Could you check a few things on this model? Use its own coordinates, in mm. A direction names the side the tool comes from. Coordinates: 2 decimals unless noted, no trailing zeros. Write each loop counter-clockwise with the first axis right and the second up, starting at its lowest first coordinate (ties: lowest second). Pieces come first, ordered by that corner, then holes.
Item 1: Thinking about a two-plate mould opening in Y: for faces 1 (the flat face through (26, 0, 25)), 2 (the flat face through (54.84, 35.87, 25.07)), 3 (the flat face through (5.823, 38.787, 24.93)), 4 (the flat face through (26, 54, 10)), which applies, +Y half, -Y half, draft (parallel to the pull), parting line (faces both ways), or undercut?
Item 2: I want a section at D-D on z = 13. Please give me the cut outline in (x, y), then the cut area to 4 significant figures.
Item 3: For P1, Ø1, axis at x = 23, z = 23, coming from the +Y side; P2, Ø4, axis at x = -9.5, z = 11, coming from the -Y side; P3, Ø4.5, axis at x = -5.5, y = 42, coming from the +Z side, each with a flat end and sliding along its axis, tell me the tip position at first contact or that it passes through.
Item 4: I want a section at B-B on x = 26. Please give me the cut outline in (y, z), then the cut area to 3 significant figures.
Item 5: If I drill on probe 1 along Z at (x, y) = (6, 42.5); probe 2 along Y at (x, z) = (50.5, 10.5); probe 3 along Y at (x, z) = (56.5, 13), over which ranges is the centre line in solid material (lowest first)?
Item 6: I want a section at A-A on z = 25. Please give me the cut outline in (x, y), then the cut area to 3 significant figures.
Item 7: I want a section at C-C on y = 32.5. Please give me the cut outline in (x, z), then the cut area to 3 significant figures.
Item 8: Which directions (+Z, -Z, +X, -X, +Y, -Y) give clear straight access to the entire face, cutting with the end or side of a thin tool? Please do faces 5 (the flat face through (26, 45, 25)), 6 (the flat face through (56, 34, 7)), 7 (the cylindrical face through (26, 45, 45)), 8 (the flat face through (-2.84, 35.87, 24.93)), 9 (the flat face through (3.5, 47, 43)).
from build123d import *

# Parameters (mm, degrees)
BASE_BLOCK_DEPTH        = 50
SADDLE_CUT_1_30_DEPTH   = 10
SADDLE_START            = -10
SADDLE_CUT_2_30_DEPTH   = 10
UPPER_BLOCK_DEPTH       = 30
UPPER_BLOCK_NOTCH_DEPTH = 20
NOTCH_PAD_1_DEPTH       = 5
NOTCH_PAD_2_DEPTH       = 5
SIDE_BLOCK_DEPTH        = 35
SIDE_BLOCK_POCKET_DEPTH = 15
TOP_HOLE_SKETCH_R       = 5
TOP_HOLE_10_DEPTH       = 15
SIDE_WINDOW_SKETCH_W    = 10
SIDE_WINDOW_SKETCH_H    = 10
SIDE_WINDOW_CUT_DEPTH   = 15
UPPER_WINDOW_SKETCH_W   = 10
UPPER_WINDOW_SKETCH_H   = 10
UPPER_WINDOW_CUT_DEPTH  = 15


with BuildPart() as part:
    # Base Profile Sketch → Base Block (new body)
    with BuildSketch(Plane.XY):
        Polygon((0, 0), (52, 0), (52, 12), (71, 12), (71, 22), (63, 34), (48, 34), (48, 60), (4, 60), (4, 34), (-11, 34), (-19, 22), (-19, 12), (0, 12), align=None)
    extrude(amount=BASE_BLOCK_DEPTH)

    # Saddle Cut 1 Sketch → Saddle Cut 1 Ø30 (cut)
    with BuildSketch(Plane.XY.offset(50)):
        with BuildLine():
            Line((11, 60), (41, 60))
            ThreePointArc((41, 60), (26, 45), (11, 60))
        make_face()
    extrude(amount=-SADDLE_CUT_1_30_DEPTH, mode=Mode.SUBTRACT)

    # Saddle Cut 2 Sketch → Saddle Cut 2 Ø30 (cut)
    with BuildSketch(Plane(origin=(0, 0, 0), x_dir=(-1, 0, 0), z_dir=(0, 0, -1)).offset(SADDLE_START)):
        with BuildLine():
            Line((-41, 60), (-11, 60))
            ThreePointArc((-11, 60), (-26, 45), (-41, 60))
        make_face()
    extrude(amount=SADDLE_CUT_2_30_DEPTH, mode=Mode.SUBTRACT)

    # Upper Block Sketch → Upper Block (add)
    with BuildSketch(Plane(origin=(0, 0, 0), x_dir=(-1, 0, 0), z_dir=(0, 0, -1))):
        Polygon((-48, 60), (-48, 34), (-63, 34), (-56, 60), align=None)
    extrude(amount=-UPPER_BLOCK_DEPTH)

    # Upper Block Notch Sketch → Upper Block Notch (cut)
    with BuildSketch(Plane(origin=(0, 0, 0), x_dir=(-1, 0, 0), z_dir=(0, 0, -1))):
        Polygon((-63, 34), (-56, 60), (-48.5, 60), (-48.5, 34), align=None)
    extrude(amount=-UPPER_BLOCK_NOTCH_DEPTH, mode=Mode.SUBTRACT)

    # Notch Pad 1 Sketch → Notch Pad 1 (add)
    with BuildSketch(Plane(origin=(0, 0, 20), x_dir=(-1, 0, 0), z_dir=(0, 0, -1))):
        Polygon((-63, 34), (-48.5, 34), (-48.5, 60), (-56, 60), align=None)
    extrude(amount=NOTCH_PAD_1_DEPTH)

    # Notch Pad 2 Sketch → Notch Pad 2 (add)
    with BuildSketch(Plane.XY.offset(30)):
        Polygon((48, 60), (56, 60), (63, 34), (48, 34), align=None)
    extrude(amount=NOTCH_PAD_2_DEPTH)

    # Side Block Sketch → Side Block (add)
    with BuildSketch(Plane.XY.offset(50)):
        Polygon((4, 60), (4, 34), (-11, 34), (-4, 60), align=None)
    extrude(amount=-SIDE_BLOCK_DEPTH)

    # Side Block Pocket Sketch → Side Block Pocket (cut)
    with BuildSketch(Plane.XY.offset(50)):
        Polygon((3.5, 60), (3.5, 34), (-11, 34), (-4, 60), align=None)
    extrude(amount=-SIDE_BLOCK_POCKET_DEPTH, mode=Mode.SUBTRACT)

    # Top Hole Sketch → Top Hole Ø10 (cut)
    with BuildSketch(Plane(origin=(0, 60, 0), x_dir=(1, 0, 0), z_dir=(0, 1, 0))):
        with Locations(Location((26, -25, 0), (0, 0, 270))):
            Circle(TOP_HOLE_SKETCH_R)
    extrude(amount=-TOP_HOLE_10_DEPTH, mode=Mode.SUBTRACT)

    # Side Window Sketch → Side Window Cut (cut)
    with BuildSketch(Plane(origin=(-18.791724138, 5.059310345, 0), x_dir=(0, 0, 1), z_dir=(-0.9656157585206698, 0.25997347344787275, 0))):
        with Locations((25, 38.897051617)):
            Rectangle(SIDE_WINDOW_SKETCH_W, SIDE_WINDOW_SKETCH_H)
    extrude(amount=-SIDE_WINDOW_CUT_DEPTH, mode=Mode.SUBTRACT)

    # Upper Window Sketch → Upper Window Cut (cut)
    with BuildSketch(Plane(origin=(67.277241379, 18.113103448, 0), x_dir=(0, 0, -1), z_dir=(0.9656157585206697, 0.2599734734478728, 0))):
        with Locations((-25, 25.378430998)):
            Rectangle(UPPER_WINDOW_SKETCH_W, UPPER_WINDOW_SKETCH_H)
    extrude(amount=-UPPER_WINDOW_CUT_DEPTH, mode=Mode.SUBTRACT)


solid = part.part
Response values:
1. face 1: -Y half
1. face 2: undercut
1. face 3: undercut
1. face 4: draft
2. outline: (-19, 12) - (0, 12) - (0, 0) - (52, 0) - (52, 12) - (71, 12) - (71, 22) - (63, 34) - (48.5, 34) - (48.5, 60) - (4, 60) - (4, 34) - (-11, 34) - (-19, 22) - close
2. area: 3,665 mm2
3. P1: stops at y = 45
3. P2: stops at y = 12
3. P3: stops at z = 35
4. outline: (0, 0) - (45, 0) - (45, 10) - (60, 10) - (60, 20) - (45, 20) - (45, 30) - (60, 30) - (60, 40) - (45, 40) - (45, 50) - (0, 50) - close
4. area: 2,550 mm2
5. probe 1: z = 0 to 20, 30 to 50
5. probe 2: y = 0 to 34
5. probe 3: y = 12 to 34
6. outline: (-19, 12) - (0, 12) - (0, 0) - (52, 0) - (52, 12) - (71, 12) - (71, 22) - (63, 34) - (61.98, 37.79) - (47.5, 33.89) - (44.9, 43.55) - (59.38, 47.45) - (56, 60) - (31, 60) - (31, 45) - (21, 45) - (21, 60) - (-4, 60) - (-7.38, 47.45) - (7.1, 43.55) - (4.5, 33.89) - (-9.98, 37.79) - (-11, 34) - (-19, 22) - close
6. area: 3,800 mm2
7. outline: (-12, 0) - (64, 0) - (64, 50) - (-12, 50) - close
7. area: 3,800 mm2
8. face 5: +Y
8. face 6: -Z, +X, +Y
8. face 7: +Z, +Y
8. face 8: none
8. face 9: +Z, -X, +Y
